Print and shaded views of the part. All mm, measured from the part's lowest x, y and z. A direction names the side the tool comes from. Coordinates: 2 decimals unless noted, no trailing zeros. Loops run counter-clockwise (first coordinate to the right, second up) from the corner with the lowest first, then second, coordinate; pieces in that order, holes last.
1) Pin check, flat tips, straight feed: pin 1 Ø25 at (x, z) = (41, 20.5) entering from +Y; pin 2 Ø3 at (y, z) = (15.5, 44.5) entering from +X. Stop position of each tip, or through.
2) Saw through at A-A, the plane z = 25. Write the cut outline in (x, y).
3) Which spindle directions (+Z, -Z, +X, -X, +Y, -Y) get a long thin tool onto all of the face, cutting with end or side? Do the marked faces 1 and 2. Say none if no direction does.
4) Wall check: line 1 along Z through (x, y) = (25, 5); line 2 along Y through (x, z) = (3.25, 41.25); line 3 along Y through (x, z) = (3, 25). Give the ranges that are in metal, low to high.
5) Saw through at C-C, the plane y = 10.5. Write the cut outline in (x, z), and give its area (3 significant figures).
6) Saw through at B-B, the plane x = 48.5. Write the cut outline in (y, z), and give its area (3 significant figures).
7) Two-plate mould, pull along Z, no slides. Class the marked faces 3, 4 and 5: +Z half, -Z half, draft (parallel to the pull), parting line (faces both ways), or undercut.
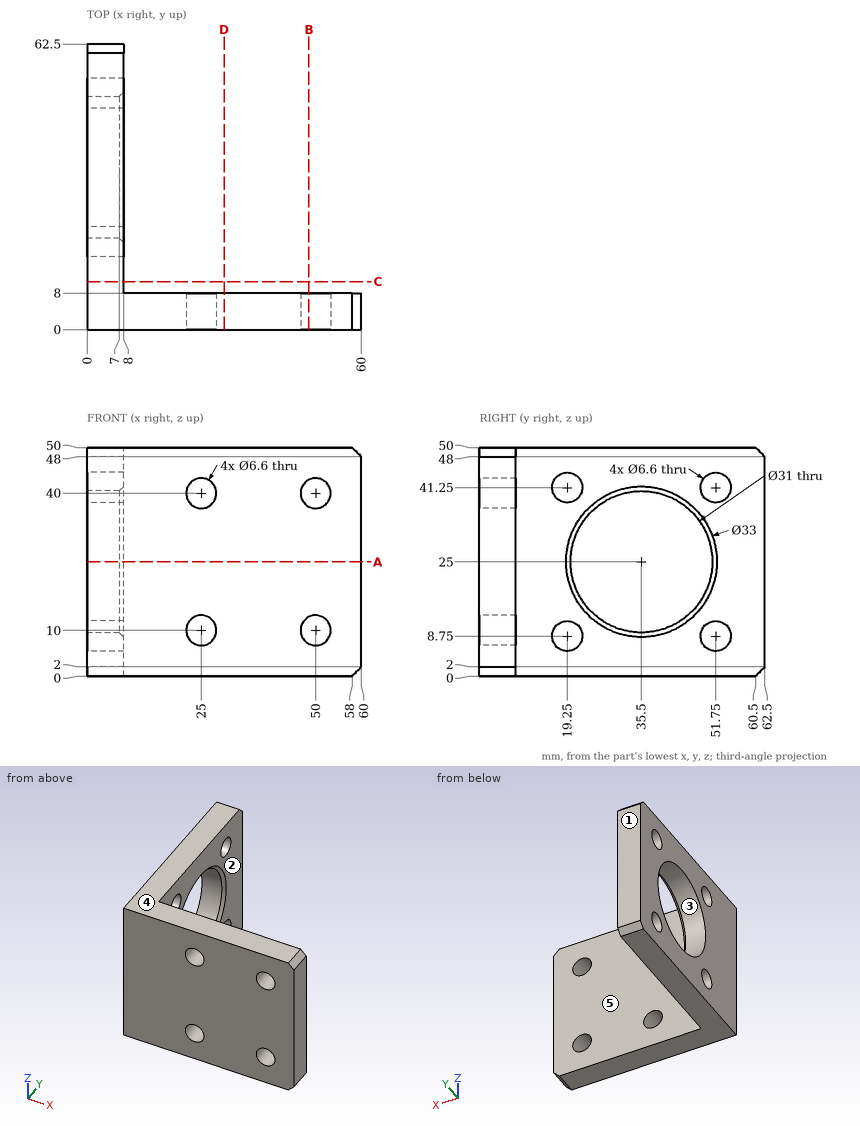
Data:
1. pin 1: stops at y = 8
1. pin 2: stops at x = 8
2. outline: (0, 0) - (60, 0) - (60, 8) - (8, 8) - (8, 19) - (7, 20) - (0, 20) - close; (0, 51) - (7, 51) - (8, 52) - (8, 62.5) - (0, 62.5) - close
3. face 1: +Z, -Z, +X, -X, +Y
3. face 2: +Z, -Z, +X, +Y
4. line 1: z = 0 to 6.7, 13.3 to 36.7, 43.3 to 50
4. line 2: y = 0 to 15.95, 22.55 to 48.45, 55.05 to 62.5
4. line 3: y = 0 to 20, 51 to 62.5
5. outline: (0, 0) - (8, 0) - (8, 50) - (0, 50) - close
5. area: 400 mm2
6. outline: (0, 0) - (8, 0) - (8, 7.06) - (0, 7.06) - close; (0, 12.94) - (8, 12.94) - (8, 37.06) - (0, 37.06) - close; (0, 42.94) - (8, 42.94) - (8, 50) - (0, 50) - close
6. area: 306 mm2
7. face 3: undercut
7. face 4: +Z half
7. face 5: draft
